Geometry: final body of the model. Coordinates: model frame, mm. A direction names the side the tool comes from. Round coordinates to 2 decimals unless told otherwise and drop trailing zeros. Loops run counter-clockwise (first coordinate to the right, second up) from the corner with the lowest first, then second, coordinate; pieces in that order, holes last. Notation, with made-up numbers: (-34, 86) -> (-18, 86) arc R30 cw to (-18, 111) -> close; hole circle Ø11 at (13.25, -28). An arc over 180 degrees is marked (long way). Answer in a Markdown table with one row per item.
```python
from build123d import *

# Parameters (mm, degrees)
BASE_BLOCK_DEPTH           = 95
UPRIGHT_BLOCK_DEPTH        = 71
UPRIGHT_CHAMFER_20X45_SIZE = 20
SLOT_RIM_BOSS_DEPTH        = 4
THROUGH_START              = -154
THROUGH_SLOT_CUT_DEPTH     = 154


with BuildPart() as part:
    # Base and Upright Profile Sketch → Base Block (new body)
    with BuildSketch(Plane(origin=(0, 0, 0), x_dir=(0, 0, -1), z_dir=(1, 0, 0))):
        Polygon((35.5, 0), (35.5, 8), (9.5, 8), (9.5, 0), (0, 0), (0, 24), (82, 24), (82, 0), align=None)
    extrude(amount=BASE_BLOCK_DEPTH)

    # Sketch1_3 → Upright Block (add)
    with BuildSketch(Plane(origin=(0, 0, 0), x_dir=(0, 0, -1), z_dir=(1, 0, 0))):
        Polygon((58, 54), (58, 71), (47, 71), (47, 24), (82, 24), (82, 71), (71, 71), (71, 54), align=None)
    extrude(amount=UPRIGHT_BLOCK_DEPTH)

    # Upright Chamfer 20x45
    upright_chamfer_20x45_edges = [part.edges().sort_by_distance(p)[0] for p in [
        (71, 71, -52.5),
    ]]
    chamfer(upright_chamfer_20x45_edges, length=UPRIGHT_CHAMFER_20X45_SIZE)

    # Slot Rim Sketch → Slot Rim Boss (add)
    with BuildSketch(Plane(origin=(0, 24, 0), x_dir=(1, 0, 0), z_dir=(0, 1, 0))):
        with BuildLine():
            Line((25, 32.5), (70, 32.5))
            ThreePointArc((70, 32.5), (81.5, 21), (70, 9.5))
            Line((70, 9.5), (25, 9.5))
            ThreePointArc((25, 9.5), (13.5, 21), (25, 32.5))
        make_face()
        with BuildLine():
            Line((25, 27.5), (70, 27.5))
            ThreePointArc((70, 27.5), (76.5, 21), (70, 14.5))
            Line((70, 14.5), (25, 14.5))
            ThreePointArc((25, 14.5), (18.5, 21), (25, 27.5))
        make_face(mode=Mode.SUBTRACT)
    extrude(amount=SLOT_RIM_BOSS_DEPTH)

    # Through Slot Sketch → Through Slot Cut (cut)
    with BuildSketch(Plane(origin=(0, 24, 0), x_dir=(1, 0, 0), z_dir=(0, 1, 0)).offset(THROUGH_START)):
        with BuildLine():
            Line((25, 27.5), (70, 27.5))
            ThreePointArc((70, 27.5), (76.5, 21), (70, 14.5))
            Line((70, 14.5), (25, 14.5))
            ThreePointArc((25, 14.5), (18.5, 21), (25, 27.5))
        make_face()
    extrude(amount=THROUGH_SLOT_CUT_DEPTH, mode=Mode.SUBTRACT)


solid = part.part
```
Item 1: Set-up query: faces 5 (the cylindrical face through (13.503, 25.972, -20.747)), 6 (the flat face through (26, 62, -58)), 7 (the flat face through (47, 4, -9.5)). Return all of +Z, -Z, +X, -X, +Y, -Y with unobstructed straight access to the full face (end or side cutting, diameter ignored); none if empty.
Ans:
| item | result |
|---|---|
| face 5 | -X, +Y |
| face 6 | +X, -X, +Y |
| face 7 | +X, -X, -Y |
Item 2: Ray query, L1, parallel to Z at x = 39.5, y = 67.5; L2, parallel to Z at x = 25, y = 13; L3, parallel to Y at x = 62, z = -41.5. Return the intervals inside material, ascending.
Ans:
| item | result |
|---|---|
| L1 | -82 to -71, -58 to -47 |
| L2 | -82 to -27.5, -14.5 to 0 |
| L3 | 0 to 24 |
Item 3: Section query D-D, the plane z = -69.5. Output: boundary loops of the cut face in (x, y).
Ans:
| item | result |
|---|---|
| outline | (0, 0) -> (95, 0) -> (95, 24) -> (71, 24) -> (71, 51) -> (68, 54) -> (0, 54) -> close |
Item 4: First-contact query: P1, Ø23.5, axis at x = 45.5, y = 45, coming from the +Z side; P2, Ø8, axis at x = 74.5, z = -14.5, coming from the +Y side; P3, Ø1, axis at x = 72.5, z = -36.5, coming from the -Y side; P4, Ø13.5, axis at y = 44, z = -58, coming from the +X side. Flat tips, straight axial feed; report the tip coordinate or a pass-through.
Ans:
| item | result |
|---|---|
| P1 | z = -47 |
| P2 | y = 28 |
| P3 | y = 0 |
| P4 | x = 71 |
Item 5: Mould query, pull axis Z, two halves, no side actions, for faces 1 (the flat face through (47, 26, -32.5)), 2 (the flat face through (47, 12, 0)), 3 (the flat face through (47, 0, -59)), 4 (the flat face through (48, 18, -14.5)). Classes: released by +Z, released by -Z, zero draft, split by the parting line, or undercut.
Ans:
| item | result |
|---|---|
| face 1 | undercut |
| face 2 | released by +Z |
| face 3 | zero draft |
| face 4 | undercut |
Item 6: Section query B-B, the plane y = 58. Output: boundary loops of the cut face in (x, z).
Ans:
| item | result |
|---|---|
| outline | (0, -82) -> (64, -82) -> (64, -71) -> (0, -71) -> close; (0, -58) -> (64, -58) -> (64, -47) -> (0, -47) -> close |
Item 7: Section query C-C, the plane y = 19.5. Output: boundary loops of the cut face in (x, z).
Ans:
| item | result |
|---|---|
| outline | (0, -82) -> (95, -82) -> (95, 0) -> (0, 0) -> close; hole (25, -27.5) -> (70, -27.5) arc R6.5 ccw to (70, -14.5) -> (25, -14.5) arc R6.5 ccw to start |
Item 8: Section query A-A, the plane z = -21. Output: boundary loops of the cut face in (x, y).
Ans:
| item | result |
|---|---|
| outline | (0, 8) -> (18.5, 8) -> (18.5, 28) -> (13.5, 28) -> (13.5, 24) -> (0, 24) -> close; (76.5, 8) -> (95, 8) -> (95, 24) -> (81.5, 24) -> (81.5, 28) -> (76.5, 28) -> close |
